Part model, mm, in its own coordinate system. A direction names the side the tool comes from. Round coordinates to 2 decimals unless told otherwise and drop trailing zeros. Loops run counter-clockwise (first coordinate to the right, second up) from the corner with the lowest first, then second, coordinate; pieces in that order, holes last. Notation, with made-up numbers: (-36, 15.5) -> (23, 15.5) arc R32 ccw to (23, 47.5) -> close; hole circle Ø8 at (-19, 15). An arc over 180 degrees is marked (long way). Use a Markdown table: item, result. Add a question column.
Item 1: Which spindle directions (+Z, -Z, +X, -X, +Y, -Y) get a long thin tool onto all of the face, cutting with end or side? Do faces 1 (the face through (-0.1, 15.2, -620)), 2 (the face through (-0.1, 15.2, 620)), 3 (the face through (6, -3, 710)). Say none if no direction does.
Item 2: Cut at A-A, the plane z = -89. List the corners of the cut face in (x, y), plus the area to 3 significant figures.
Item 3: Probe line 1 (Y direction, x = 0, z = 698); line 2 (Z direction, x = -11, y = -14.5); line 3 (Y direction, x = 13, z = -76). List the from-to ranges inside material, lowest first. Write a range as [from, to].
Item 4: Flat gauge pins, fed straight in: pin 1 (1 mm diameter, centred on x = -2.5, z = 436.5, fed in from +Y); pin 2 (8 mm diameter, centred on x = 0.5, z = -564, fed in from -Y); pin 3 (3 mm diameter, centred on x = 13, z = 482, fed in from -Y). Where does each tip first touch, or does it go through?
```python
from build123d import *

# Parameters (mm, degrees)
SKETCH1_R              = 15
BOSS_EXTRUDE1_DEPTH    = 710
M14_TAPPED_HOLE2_D     = 12
M14_TAPPED_HOLE2_DEPTH = 34
M14_TAPPED_HOLE2_TIP   = 3.605163714
M14_TAPPED_HOLE1_D     = 12
M14_TAPPED_HOLE1_DEPTH = 34
M14_TAPPED_HOLE1_TIP   = 3.605163714
SKETCH7_R              = 20
BOSS_EXTRUDE3_DEPTH    = 620
CHAMFER1_SIZE          = 1.5


with BuildPart() as part:
    # Sketch1 → Boss-Extrude1 (new, symmetric)
    with BuildSketch(Plane.XY):
        Circle(SKETCH1_R)
    extrude(amount=BOSS_EXTRUDE1_DEPTH, both=True)

    # M14 Tapped Hole2
    with Locations(Plane.XY.offset(710)):
        with Locations((0, 0)):
            Hole(M14_TAPPED_HOLE2_D / 2, depth=M14_TAPPED_HOLE2_DEPTH)
            with Locations((0, 0, -(M14_TAPPED_HOLE2_DEPTH + M14_TAPPED_HOLE2_TIP / 2))):  # 118° drill point
                Cone(0, M14_TAPPED_HOLE2_D / 2, M14_TAPPED_HOLE2_TIP, mode=Mode.SUBTRACT)

    # M14 Tapped Hole1
    with Locations(Plane(origin=(0, 0, -710), x_dir=(-1, 0, 0), z_dir=(0, 0, -1))):
        with Locations((0, 0)):
            Hole(M14_TAPPED_HOLE1_D / 2, depth=M14_TAPPED_HOLE1_DEPTH)
            with Locations((0, 0, -(M14_TAPPED_HOLE1_DEPTH + M14_TAPPED_HOLE1_TIP / 2))):  # 118° drill point
                Cone(0, M14_TAPPED_HOLE1_D / 2, M14_TAPPED_HOLE1_TIP, mode=Mode.SUBTRACT)

    # Sketch7 → Boss-Extrude3 (add, symmetric)
    with BuildSketch(Plane.XY):
        Circle(SKETCH7_R)
    extrude(amount=BOSS_EXTRUDE3_DEPTH, both=True)

    # Chamfer1
    chamfer1_edges = [part.edges().sort_by_distance(p)[0] for p in [
        (-20, 0, -620),
        (-20, 0, 620),
        (-15, 0, -710),
        (-15, 0, 710),
    ]]
    chamfer(chamfer1_edges, length=CHAMFER1_SIZE)


solid = part.part
```
A:
| question | item | result |
|---|---|---|
| 1 | face 1 | -Z |
| 1 | face 2 | +Z |
| 1 | face 3 | +Z, +X, -X, +Y, -Y |
| 2 | outline | circle Ø40 at (0, 0) |
| 2 | area | 1,260 mm^2 |
| 3 | line 1 | y = [-15, -6], [6, 15] |
| 3 | line 2 | z = [-620, 620] |
| 3 | line 3 | y = [-15.2, 15.2] |
| 4 | pin 1 | stops at y = 19.9 |
| 4 | pin 2 | stops at y = -20 |
| 4 | pin 3 | stops at y = -16.36 |
